CAD build for the part. Positions are in the model's coordinates, mm. A direction names the side the tool comes from. Coordinates: 2 decimals unless noted, no trailing zeros. Loops run counter-clockwise (first coordinate to the right, second up) from the corner with the lowest first, then second, coordinate; pieces in that order, holes last. Notation, with made-up numbers: (52, 39.25) -> (111, 39.25) arc R33 ccw to (111, 69.25) -> close; hole circle Ø10 at (-17, 83.5). An arc over 180 degrees is marked (long way). Write item = value, one per line. Start each with the question number.
(1) Band-saw the part on A-A (y = 15). Write the cut outline in (x, z), and give its area (3 significant figures).
(2) Drill centre lines: line 1 (X direction, y = 19, z = 60); line 2 (Z direction, x = 0, y = 19.25); line 3 (X direction, y = 21, z = -6). Where is each one in solid material? Low to high. Write a range as from..to.
(3) Pull direction Z, two halves, no side cores. Call faces 1 (the face through (84.41, 5.605, 59.974)), 2 (the face through (-1, 25, -51)), 3 (the face through (-1, 12, -75)), 4 (the face through (-1, 12, 75)): +Z half, -Z half, draft (parallel to the pull), parting line (faces both ways), or undercut.
(4) Band-saw the part on C-C (z = 4.5). Write the cut outline in (x, y).
(5) Flat gauge pin, fed straight in: P1, Ø6, axis at x = -85, z = -60, coming from the +Y side. Where does the tip first touch, or does it go through?
(6) Tool access for faces 5 (the face through (100, 12, 1)), 6 (the face through (0.74, 15.71, -56.68)), 7 (the face through (-70, 12, 1)): list every direction of +Z, -Z, +X, -X, +Y, -Y with a clear straight run to the whole face (end or side of a thin tool).
(7) Band-saw the part on B-B (x = -10.5). Write the cut outline in (y, z).
```python
from build123d import *

# Parameters (mm, degrees)
SKETCH_1_W                   = 200
SKETCH_1_H                   = 150
EXTRUDE_1_DEPTH              = 25
HOLE_WIZARD_M8_1_D           = 6.8
HOLE_WIZARD_M8_1_DEPTH       = 17.707073895
HOLE_WIZARD_M8_1_CSINK_D     = 8.05
HOLE_WIZARD_M8_1_CSINK_ANGLE = 90
HOLE_WIZARD_M8_1_TIP         = 2.042926105
CUT_EXTRUDE_1_DEPTH          = 128.47548784
CUT_EXTRUDE_1_DEPTH_BACK     = 128.47548784
SKETCH_5_W                   = 140
SKETCH_5_H                   = 90


with BuildPart() as part:
    # 草图1 → 凸台-拉伸1 (new body)
    with BuildSketch(Plane(origin=(0, 0, 0), x_dir=(1, 0, 0), z_dir=(0, 1, 0))):
        Rectangle(SKETCH_1_W, SKETCH_1_H)
    extrude(amount=EXTRUDE_1_DEPTH)

    # M8 螺纹孔1
    with Locations(Plane(origin=(0, 25, 0), x_dir=(1, 0, 0), z_dir=(0, 1, 0))):
        with Locations((-85, -60), (0, -60), (85, -60), (85, 60), (0, 60), (-85, 60)):
            CounterSinkHole(HOLE_WIZARD_M8_1_D / 2, HOLE_WIZARD_M8_1_CSINK_D / 2, depth=HOLE_WIZARD_M8_1_DEPTH, counter_sink_angle=HOLE_WIZARD_M8_1_CSINK_ANGLE)
            with Locations((0, 0, -(HOLE_WIZARD_M8_1_DEPTH + HOLE_WIZARD_M8_1_TIP / 2))):  # 118° drill point
                Cone(0, HOLE_WIZARD_M8_1_D / 2, HOLE_WIZARD_M8_1_TIP, mode=Mode.SUBTRACT)

    # 草图5 → 切除-拉伸1 (cut, two sides: drawn at the far end of the back side and taken through both)
    with BuildSketch(Plane(origin=(0, 25, 0), x_dir=(1, 0, 0), z_dir=(0, 1, 0)).offset(-CUT_EXTRUDE_1_DEPTH_BACK)):
        Rectangle(SKETCH_5_W, SKETCH_5_H)
    extrude(amount=CUT_EXTRUDE_1_DEPTH + CUT_EXTRUDE_1_DEPTH_BACK, mode=Mode.SUBTRACT)


solid = part.part
```
Findings below:
q1.outline = (-100, -75) -> (100, -75) -> (100, 75) -> (-100, 75) -> close; hole circle Ø6.8 at (-85, -60); hole circle Ø6.8 at (-85, 60); hole (-70, -45) -> (70, -45) -> (70, 45) -> (-70, 45) -> close; hole circle Ø6.8 at (0, -60); hole circle Ø6.8 at (0, 60); hole circle Ø6.8 at (85, -60); hole circle Ø6.8 at (85, 60)
q1.area = 17,200 mm²
q2.line_1 = -100..-88.4, -81.6..-3.4, 3.4..81.6, 88.4..100
q2.line_2 = -75..-63.4, -56.6..-45, 45..56.6, 63.4..75
q2.line_3 = -100..-70, 70..100
q3.face_1 = undercut
q3.face_2 = draft
q3.face_3 = -Z half
q3.face_4 = +Z half
q4.outline = (-100, 0) -> (-70, 0) -> (-70, 25) -> (-100, 25) -> close; (70, 0) -> (100, 0) -> (100, 25) -> (70, 25) -> close
q5.P1 = 7.05
q6.face_5 = +Z, -Z, +X, +Y, -Y
q6.face_6 = +Y
q6.face_7 = +Y, -Y
q7.outline = (0, -75) -> (25, -75) -> (25, -45) -> (0, -45) -> close; (0, 45) -> (25, 45) -> (25, 75) -> (0, 75) -> close
